Geometry check sheet. Reference: drawing and pictorial views, mm from the part's lowest x, y, z. Coordinates: 2 decimals unless noted, no trailing zeros. Write each loop counter-clockwise with the first axis right and the second up, starting at its lowest first coordinate (ties: lowest second). Pieces come first, ordered by that corner, then holes. Notation, with made-up numbers: (12, -26.75) -> (26, -26.75) arc R21 ccw to (26, -11.75) -> close; hole circle Ø11 at (26, -23.5). An arc over 180 degrees is marked (long way). Use a Markdown table: item, result.
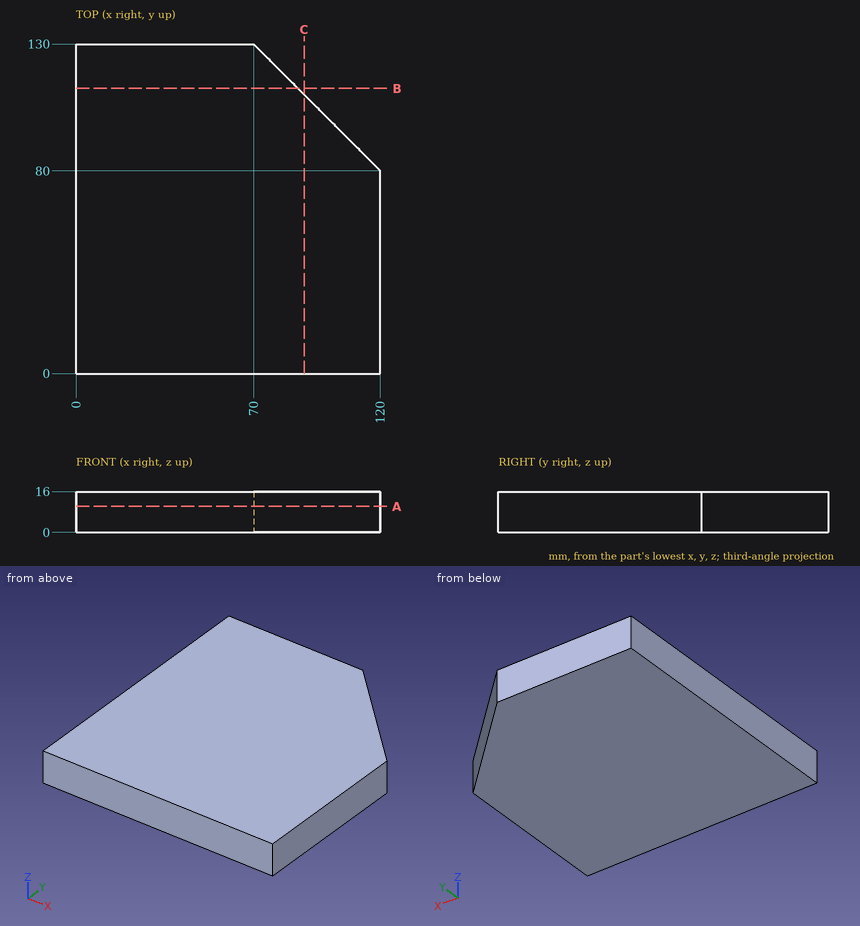
Item 1: Section check C-C on x = 90. Record the boundary of the cut face in (y, z).
Answer block:
| item | result |
|---|---|
| outline | (0, 0) -> (110, 0) -> (110, 16) -> (0, 16) -> close |
Item 2: Thickness scan on L1, parallel to X at y = 90, z = 12.25; L2, parallel to X at y = 88.5, z = 5; L3, parallel to Y at x = 105.5, z = 11. Record the ranges inside material, lowest first. Write a range as [from, to].
Answer block:
| item | result |
|---|---|
| L1 | x = [0, 110] |
| L2 | x = [0, 111.5] |
| L3 | y = [0, 94.5] |
Item 3: Depth check by flat-ended pin: P1, Ø8, axis at x = 82, z = 5, coming from the +Y side; P2, Ø3, axis at y = 109.5, z = 3.5, coming from the +X side; P3, Ø1.5, axis at y = 96.5, z = 2.5, coming from the +X side. Enter the tip coordinate at first touch or a pass-through.
Answer block:
| item | result |
|---|---|
| P1 | stops at y = 122 |
| P2 | stops at x = 92 |
| P3 | stops at x = 104.25 |
Item 4: Section check A-A on z = 10.25. Record the boundary of the cut face in (x, y).
Answer block:
| item | result |
|---|---|
| outline | (0, 0) -> (120, 0) -> (120, 80) -> (70, 130) -> (0, 130) -> close |
Item 5: Section check B-B on y = 112.5. Record the boundary of the cut face in (x, z), then the cut area to 3 significant figures.
Answer block:
| item | result |
|---|---|
| outline | (0, 0) -> (87.5, 0) -> (87.5, 16) -> (0, 16) -> close |
| area | 1,400 mm^2 |
